Here's how the part is built. I have some questions about the finished solid (model axes, mm). Face numbers are marked on the shaded views. A direction names the side the tool comes from. Give positions to 0.01 mm unless a question says otherwise; leave off trailing zeros. Loops run counter-clockwise (first coordinate to the right, second up) from the corner with the lowest first, then second, coordinate; pieces in that order, holes last. Notation, with made-up numbers: (62.25, -33.5) - (79.25, -33.5) arc R17 ccw to (79.25, -0.5) - close; hole circle Ø11 at (-9.5, 45). An arc over 180 degrees is marked (long way). One line per item, written item: value. Start each with the question number.
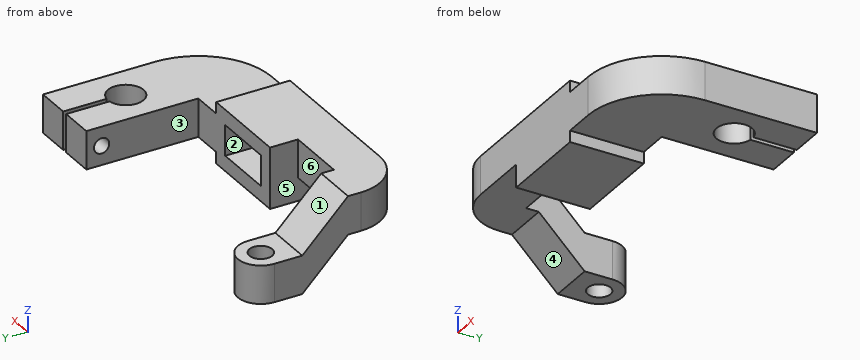
```python
from build123d import *

# Parameters (mm, degrees)
BASE_BODY_DEPTH             = 15
ARM_BLOCK_DEPTH             = 18
INCLINED_ARM_SKETCH_W       = 15
INCLINED_ARM_SKETCH_H       = 11
INCLINED_ARM_DEPTH          = 18
TOP_LUG_DEPTH               = 15
LUG_HOLE_SKETCH_R           = 4.5
LUG_HOLE_9_DEPTH            = 15
POCKET_BOSS_SKETCH_W        = 36
POCKET_BOSS_SKETCH_H        = 29
POCKET_BOSS_DEPTH           = 9
CLEVIS_BLOCK_SKETCH_W       = 12
CLEVIS_BLOCK_SKETCH_H       = 15
CLEVIS_BLOCK_DEPTH          = 29
CLEVIS_CORNER_DEPTH         = 15
CLEVIS_JAW_DEPTH            = 15
CLEVIS_HOLE_SKETCH_R        = 7
CLEVIS_HOLE_14_DEPTH        = 15
CLEVIS_SLOT_DEPTH           = 18
JAW_HOLE_SKETCH_R           = 3
JAW_HOLE_6_DEPTH            = 15
RECTANGULAR_POCKET_SKETCH_W = 24
RECTANGULAR_POCKET_SKETCH_H = 12
RECTANGULAR_POCKET_DEPTH    = 18


with BuildPart() as part:
    # Base Profile Sketch → Base Body (new body)
    with BuildSketch(Plane.XY):
        with BuildLine():
            Line((0, -18), (60, -18))
            Line((60, -18), (60, 11))
            Line((60, 11), (24, 11))
            Line((24, 11), (24, 0))
            Line((24, 0), (0, 0))
            Line((0, 0), (0, 5))
            Line((0, 5), (-18, 5))
            Line((-18, 5), (-18, 0))
            ThreePointArc((-18, 0), (-12.727922061, -12.727922061), (0, -18))
        make_face()
    extrude(amount=BASE_BODY_DEPTH)

    # Arm Block Sketch → Arm Block (add)
    with BuildSketch(Plane.ZY.offset(18)):
        Polygon((-18, 23), (-3, 23), (15, 5), (0, 5), align=None)
    extrude(amount=-ARM_BLOCK_DEPTH)

    # Inclined Arm Sketch → Inclined Arm (add)
    with BuildSketch(Plane.ZY.offset(18)):
        with Locations((-10.5, 28.5)):
            Rectangle(INCLINED_ARM_SKETCH_W, INCLINED_ARM_SKETCH_H)
    extrude(amount=-INCLINED_ARM_DEPTH)

    # Top Lug Sketch → Top Lug (add)
    with BuildSketch(Plane.XY.offset(-3)):
        with BuildLine():
            Line((-18, 34), (0, 34))
            ThreePointArc((0, 34), (-9, 43), (-18, 34))
        make_face()
    extrude(amount=-TOP_LUG_DEPTH)

    # Lug Hole Sketch → Lug Hole Ø9 (cut)
    with BuildSketch(Plane.XY.offset(-3)):
        with Locations((-9, 34)):
            Circle(LUG_HOLE_SKETCH_R)
    extrude(amount=-LUG_HOLE_9_DEPTH, mode=Mode.SUBTRACT)

    # Pocket Boss Sketch → Pocket Boss (add)
    with BuildSketch(Plane(origin=(0, 0, 0), x_dir=(-1, 0, 0), z_dir=(0, 0, -1))):
        with Locations((-42, -3.5)):
            Rectangle(POCKET_BOSS_SKETCH_W, POCKET_BOSS_SKETCH_H)
    extrude(amount=POCKET_BOSS_DEPTH)

    # Clevis Block Sketch → Clevis Block (add)
    with BuildSketch(Plane(origin=(0, 11, 0), x_dir=(1, 0, 0), z_dir=(0, 1, 0))):
        with Locations((66, -3)):
            Rectangle(CLEVIS_BLOCK_SKETCH_W, CLEVIS_BLOCK_SKETCH_H)
    extrude(amount=-CLEVIS_BLOCK_DEPTH)

    # Clevis Corner Sketch → Clevis Corner (add)
    with BuildSketch(Plane.XY.offset(10.5)):
        with BuildLine():
            Line((72, 11), (101, 11))
            ThreePointArc((101, 11), (92.506096654, -9.506096654), (72, -18))
            Line((72, -18), (72, 11))
        make_face()
    extrude(amount=-CLEVIS_CORNER_DEPTH)

    # Clevis Jaw Sketch → Clevis Jaw (add)
    with BuildSketch(Plane.XY.offset(10.5)):
        Polygon((101, 11), (72, 11), (72, 31), (72, 55), (101, 55), align=None)
    extrude(amount=-CLEVIS_JAW_DEPTH)

    # Clevis Hole Sketch → Clevis Hole Ø14 (cut)
    with BuildSketch(Plane.XY.offset(10.5)):
        with Locations((86.5, 31)):
            Circle(CLEVIS_HOLE_SKETCH_R)
    extrude(amount=-CLEVIS_HOLE_14_DEPTH, mode=Mode.SUBTRACT)

    # Clevis Slot Sketch → Clevis Slot (cut)
    with BuildSketch(Plane(origin=(0, 55, 0), x_dir=(1, 0, 0), z_dir=(0, 1, 0))):
        Polygon((86.5, 4.5), (85.5, 4.5), (85.5, -10.5), (87.5, -10.5), (87.5, 4.5), align=None)
    extrude(amount=-CLEVIS_SLOT_DEPTH, mode=Mode.SUBTRACT)

    # Jaw Hole Sketch → Jaw Hole Ø6 (cut)
    with BuildSketch(Plane.ZY.offset(-72)):
        with Locations((3, 49)):
            Circle(JAW_HOLE_SKETCH_R)
    extrude(amount=-JAW_HOLE_6_DEPTH, mode=Mode.SUBTRACT)

    # Rectangular Pocket Sketch → Rectangular Pocket (cut)
    with BuildSketch(Plane(origin=(0, 11, 0), x_dir=(1, 0, 0), z_dir=(0, 1, 0))):
        with Locations((42, -3)):
            Rectangle(RECTANGULAR_POCKET_SKETCH_W, RECTANGULAR_POCKET_SKETCH_H)
    extrude(amount=-RECTANGULAR_POCKET_DEPTH, mode=Mode.SUBTRACT)


solid = part.part
```
(1) If we section it at C-C on y = 49: List the corners of the cut face in (x, z) for me.
(2) If we section it at B-B on z = 3: List the corners of the cut face in (x, y) for me, plus the area to 3 significant figures.
(3) Will these pins go through, and if not, where does the flat tip stop? pin 1 (2 mm diameter, centred on y = 42.5, z = -5, fed in from -X); pin 2 (9.5 mm diameter, centred on y = -0.5, z = 5, fed in from +X); pin 3 (16.5 mm diameter, centred on x = 15, z = 6.5, fed in from +Y).
(4) If we section it at A-A on y = 19: List the corners of the cut face in (x, z) for me, plus the area to 3 significant figures.
(5) For the marked faces 4, 5 and 6, which set-ups out of +Z, -Z, +X, -X, +Y, -Y let a thin tool reach every point of the face, with its end or its side?
(6) If we mould it in two halves opening along Z, with no side actions, what happens to the marked faces 1, 2 and 3? For each: pulls with the +Z half, pulls with the -Z half, needs draft (parallel to the pull), parting line crosses it, or undercut.
(7) Please list where these lines run through material, in increasing order: probe 1 along X at (y, z) = (14.5, 1.5); probe 2 along X at (y, z) = (41, 6.5); probe 3 along Z at (x, y) = (41.5, 1.5). Write a range as from..to.
(8) If we section it at D-D on x = -9: List the corners of the cut face in (y, z) for me.
Found:
1. outline: (72, -4.5) - (85.5, -4.5) - (85.5, 0) - (72, 0) - close; (72, 6) - (85.5, 6) - (85.5, 10.5) - (72, 10.5) - close; (87.5, -4.5) - (101, -4.5) - (101, 10.5) - (87.5, 10.5) - close
2. outline: (-18, 0) arc R18 ccw to (0, -18) - (72, -18) arc R29 ccw to (101, 11) - (101, 55) - (87.5, 55) - (87.5, 37.93) arc R7 cw (long way) to (85.5, 37.93) - (85.5, 46) - (72, 46) - (72, 11) - (54, 11) - (54, -7) - (30, -7) - (30, 11) - (24, 11) - (24, 0) - (0, 0) - (0, 17) - (-18, 17) - close; (72, 52) - (85.5, 52) - (85.5, 55) - (72, 55) - close
2. area: 3,620 mm^2
3. pin 1: x = -13.97
3. pin 2: x = 100.2
3. pin 3: y = 0
4. outline: (-18, -14) - (0, -14) - (0, 1) - (-18, 1) - close; (72, -4.5) - (101, -4.5) - (101, 10.5) - (72, 10.5) - close
4. area: 705 mm^2
5. face 4: -Z, -X, -Y
5. face 5: -Z, +Y
5. face 6: +Z, -Z, +Y
6. face 1: pulls with the +Z half
6. face 2: undercut
6. face 3: needs draft
7. probe 1: -18..0, 72..101
7. probe 2: 72..85.5, 87.5..101
7. probe 3: -9..-3, 9..15
8. outline: (-15.59, 0) - (5, 0) - (23, -18) - (29.5, -18) - (29.5, -3) - (23, -3) - (5, 15) - (-15.59, 15) - close; (38.5, -18) - (43, -18) - (43, -3) - (38.5, -3) - close
